Verification items for the finished model (mm, model axes). Face numbers are marked on the shaded views. A direction names the side the tool comes from. Coordinates: 2 decimals unless noted, no trailing zeros. Order: outer loops, then holes, each group sorted by start corner. A loop starts at its lowest first (then second) coordinate and runs counter-clockwise, first axis right, second up.
Q1. Depth check by flat-ended pin: P1, Ø1.5, axis at y = 3.5, z = -1, coming from the +X side; P2, Ø0.9, axis at x = 0, y = 7, coming from the +Z side. Enter the tip coordinate at first touch or a pass-through.
Q2. Set-up check for the marked faces 1, 2 and 3: record each of +Z, -Z, +X, -X, +Y, -Y from which the full face is reachable in a straight line by a thin tool's end or side.
Q3. Cross-section at B-B, the plane z = 0. Record the boundary of the cut face in (x, y), and give its area (3 significant figures).
Q4. Cross-section at D-D, the plane y = 2. Record the boundary of the cut face in (x, z), and give its area (3 significant figures).
Q5. Cross-section at A-A, the plane x = 0. Record the boundary of the cut face in (y, z), and give its area (3 significant figures).
Q6. Cross-section at C-C, the plane y = 11.75. Record the boundary of the cut face in (x, z).
Q7. Thickness scan on line 1 (X direction, y = 13.25, z = 0); line 2 (Y direction, x = 2.5, z = -1); line 3 (Z direction, x = -1.25, y = 15.5). Record the ranges inside material, lowest first.
from build123d import *

# Parameters (mm, degrees)
SKETCH1_R           = 2.5
BOSS_EXTRUDE1_DEPTH = 15
SKETCH2_R           = 3.25
BOSS_EXTRUDE2_DEPTH = 2
CHAMFER1_SIZE       = 0.5
CHAMFER2_SIZE       = 0.3
SKETCH3_W           = 5.914103074
SKETCH3_H           = 1
CUT_EXTRUDE1_DEPTH  = 10


with BuildPart() as part:
    # Sketch1 → Boss-Extrude1 (new body)
    with BuildSketch(Plane(origin=(0, 0, 0), x_dir=(1, 0, 0), z_dir=(0, 1, 0))):
        with Locations(Location((0, 0, 0), (0, 0, 270))):
            Circle(SKETCH1_R)
    extrude(amount=BOSS_EXTRUDE1_DEPTH)

    # Sketch2 → Boss-Extrude2 (add)
    with BuildSketch(Plane(origin=(0, 15, 0), x_dir=(1, 0, 0), z_dir=(0, 1, 0))):
        with Locations(Location((0, 0, 0), (0, 0, 270))):
            Circle(SKETCH2_R)
    extrude(amount=BOSS_EXTRUDE2_DEPTH)

    # Chamfer1
    chamfer1_edges = [part.edges().sort_by_distance(p)[0] for p in [
        (0, 17, -3.25),
    ]]
    chamfer(chamfer1_edges, length=CHAMFER1_SIZE)

    # Chamfer2
    chamfer2_edges = [part.edges().sort_by_distance(p)[0] for p in [
        (0, 0, -2.5),
    ]]
    chamfer(chamfer2_edges, length=CHAMFER2_SIZE)

    # Sketch3 → Cut-Extrude1 (cut)
    with BuildSketch(Plane.XZ):
        with Locations((0, 2.5)):
            Rectangle(SKETCH3_W, SKETCH3_H)
    extrude(amount=-CUT_EXTRUDE1_DEPTH, mode=Mode.SUBTRACT)


solid = part.part
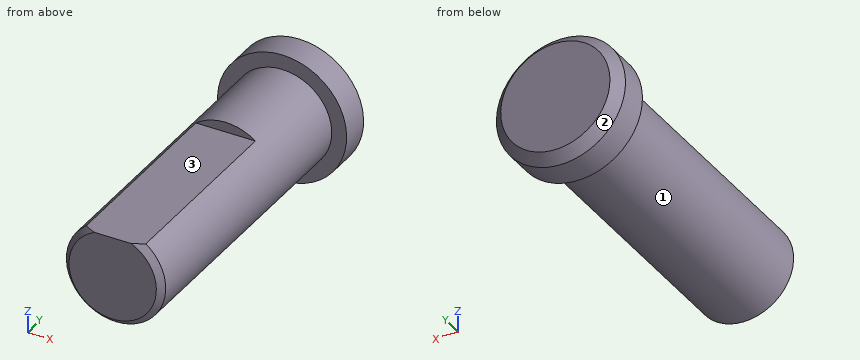
Check values:
1. P1: stops at x = 2.49
1. P2: stops at z = 2
2. face 1: -Y
2. face 2: +Y
2. face 3: +Z, +X, -X, -Y
3. outline: (-3.25, 15) - (-2.5, 15) - (-2.5, 0.3) - (-2.2, 0) - (2.2, 0) - (2.5, 0.3) - (2.5, 15) - (3.25, 15) - (3.25, 16.5) - (2.75, 17) - (-2.75, 17) - (-3.25, 16.5) - close
3. area: 87.7 mm2
4. outline: (-1.5, 2) arc R2.5 ccw (long way) to (1.5, 2) - close
4. area: 18.6 mm2
5. outline: (0, -2.2) - (0.3, -2.5) - (15, -2.5) - (15, -3.25) - (16.5, -3.25) - (17, -2.75) - (17, 2.75) - (16.5, 3.25) - (15, 3.25) - (15, 2.5) - (10, 2.5) - (10, 2) - (0, 2) - close
5. area: 82.7 mm2
6. outline: circle Ø5 at (0, 0)
7. line 1: x = -2.5 to 2.5
7. line 2: y = 15 to 17
7. line 3: z = -3 to 3
